Print and shaded views of the part. All mm, measured from the part's lowest x, y and z. Coordinates: 2 decimals unless noted, no trailing zeros. Order: outer loops, then holes, each group sorted by start corner. A loop starts at its lowest first (then second) coordinate and runs counter-clockwise, first axis right, second up. Notation, with made-up numbers: M 78.25,-16 L 135.25,-16 A31 ccw 135.25,16 Z; hole C -24,33 d11. An arc over 180 degrees is marked long. Return JSON: item names as keys, results as strings.
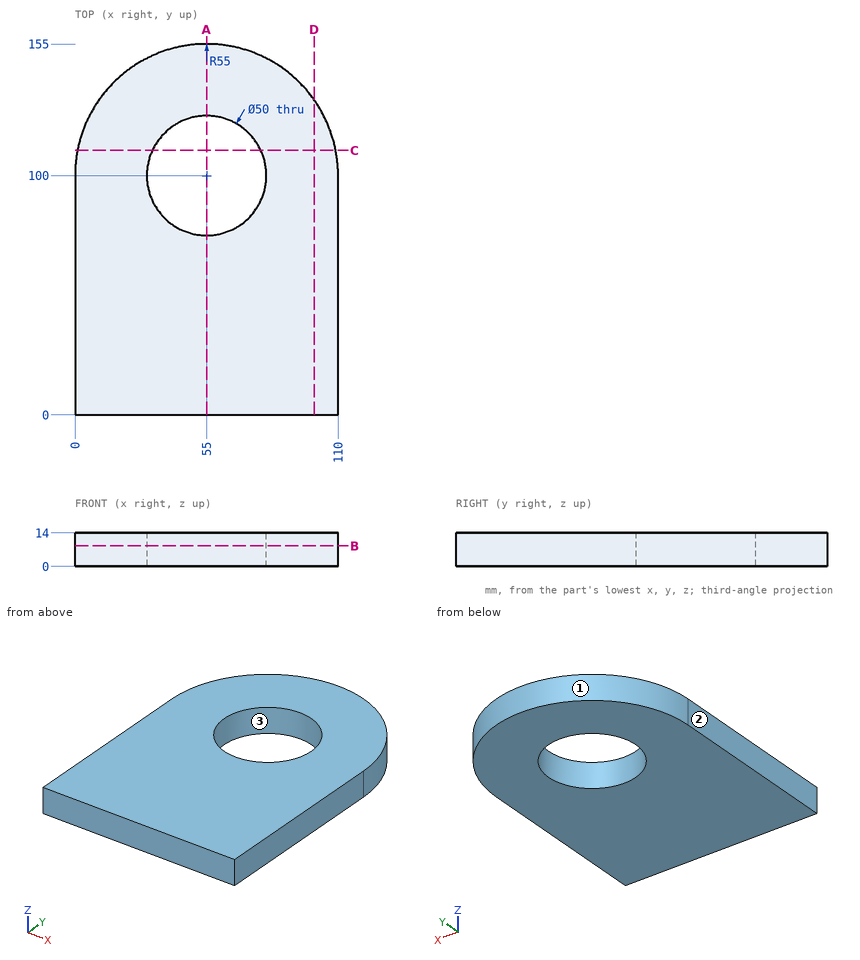
Item 1: Saw through at D-D (x = 100). Write the cut outline in (y, z), and give its area (3 significant figures).
Check result:
{"outline": "M 0,0 L 131.62,0 L 131.62,14 L 0,14 Z", "area": "1,840 mm2"}
Item 2: Saw through at C-C (y = 110.5). Write the cut outline in (x, z).
Check result:
{"outline": "M 1.01,0 L 32.31,0 L 32.31,14 L 1.01,14 Z; M 77.69,0 L 108.99,0 L 108.99,14 L 77.69,14 Z"}
Item 3: Saw through at B-B (z = 8.5). Write the cut outline in (x, y), and give its area (3 significant figures).
Check result:
{"outline": "M 0,0 L 110,0 L 110,100 A55 ccw 0,100 Z; hole C 55,100 d50", "area": "13,800 mm2"}
Item 4: Wall check: line 1 (Y direction, x = 55, z = 7.75); line 2 (X direction, y = 99.5, z = 1.75) (3 decimals); line 3 (X direction, y = 149, z = 9). Give the ranges that are in metal, low to high.
Check result:
{"line 1": "y = 0 to 75, 125 to 155", "line 2": "x = 0 to 30.005, 79.995 to 110", "line 3": "x = 30.02 to 79.98"}
Item 5: Pull direction Y, two halves, no side cores. Call the marked faces 1, 2 and 3: +Y half, -Y half, draft (parallel to the pull), parting line (faces both ways), or undercut.
Check result:
{"face 1": "+Y half", "face 2": "draft", "face 3": "undercut"}
Item 6: Saw through at A-A (x = 55). Write the cut outline in (y, z), and give its area (3 significant figures).
Check result:
{"outline": "M 0,0 L 75,0 L 75,14 L 0,14 Z; M 125,0 L 155,0 L 155,14 L 125,14 Z", "area": "1,470 mm2"}
Item 7: Drop a flat-ended pin along its axis: pin 1 Ø1.5 at (x, z) = (80, 3) entering from +Y. Give the stop position or say it passes through.
Check result:
{"pin 1": "stops at y = 149.37"}
